Build history of the part. All positions in model axes, mm. A direction names the side the tool comes from. Round coordinates to 2 decimals unless told otherwise and drop trailing zeros. Loops run counter-clockwise (first coordinate to the right, second up) from the corner with the lowest first, then second, coordinate; pieces in that order, holes last.
from build123d import *

# Parameters (mm, degrees)
SKETCH1_R           = 5
SKETCH1_R_2         = 1.5
BOSS_EXTRUDE1_DEPTH = 3
BOSS_EXTRUDE2_START = -3
BOSS_EXTRUDE2_DEPTH = 3
CUT_EXTRUDE2_DEPTH  = 65.81382707
CUT_EXTRUDE3_START  = -10
CUT_EXTRUDE3_DEPTH  = 10


with BuildPart() as part:
    # Sketch1 → Boss-Extrude1 (new body)
    # profile 1 of 3: a face of its own
    with BuildSketch(Plane(origin=(0, 0, 0), x_dir=(0, 0, -1), z_dir=(1, 0, 0))):
        with Locations((5, 5)):
            Circle(SKETCH1_R)
        with Locations((5, 5)):
            Circle(SKETCH1_R_2, mode=Mode.SUBTRACT)
    # profile 2 of 3: a face of its own
    with BuildSketch(Plane(origin=(0, 0, 0), x_dir=(0, 0, -1), z_dir=(1, 0, 0))):
        with BuildLine():
            ThreePointArc((10, 5), (8.535533906, 1.464466094), (5, 0))
            Line((5, 0), (27, 0))
            ThreePointArc((27, 0), (22, 5), (27, 10))
            Line((27, 10), (5, 10))
            ThreePointArc((5, 10), (8.535533906, 8.535533906), (10, 5))
        make_face()
    # profile 3 of 3: a face of its own
    with BuildSketch(Plane(origin=(0, 0, 0), x_dir=(0, 0, -1), z_dir=(1, 0, 0))):
        with Locations((27, 5)):
            Circle(SKETCH1_R)
        with Locations((27, 5)):
            Circle(SKETCH1_R_2, mode=Mode.SUBTRACT)
    extrude(amount=BOSS_EXTRUDE1_DEPTH)

    # Sketch2 → Boss-Extrude2 (add)
    with BuildSketch(Plane(origin=(3, 0, 0), x_dir=(0, 0, -1), z_dir=(1, 0, 0)).offset(BOSS_EXTRUDE2_START)):
        with BuildLine():
            ThreePointArc((27, 10), (29.694507461, 9.21184396), (31.53953799, 7.095851816))
            Line((31.53953799, 7.095851816), (31.610157793, 7.262674791))
            Line((31.610157793, 7.262674791), (44.585599673, 12.519851602))
            Line((44.585599673, 12.519851602), (51.097249205, 9.763328363))
            Line((51.097249205, 9.763328363), (60.365421977, 13.518454657))
            Line((60.365421977, 13.518454657), (56.610295683, 22.786627428))
            Line((56.610295683, 22.786627428), (25.051124858, 10))
            Line((25.051124858, 10), (27, 10))
        make_face()
        Polygon((60.365421977, 13.518454657), (51.097249205, 9.763328363), (51.333822162, 9.179433479), (60.601994933, 12.934559772), align=None)
    extrude(amount=BOSS_EXTRUDE2_DEPTH)

    # Sketch4 → Cut-Extrude2 (cut, through all)
    with BuildSketch(Plane(origin=(3, 0, 0), x_dir=(0, 0, -1), z_dir=(1, 0, 0))):
        Polygon((56.610295683, 22.786627428), (51.684261855, 20.790777803), (58.606145308, 17.8605936), align=None)
    extrude(amount=-CUT_EXTRUDE2_DEPTH, mode=Mode.SUBTRACT)

    # Sketch5 → Cut-Extrude3 (cut)
    with BuildSketch(Plane(origin=(3, 0, 0), x_dir=(0, 0, -1), z_dir=(1, 0, 0)).offset(CUT_EXTRUDE3_START)):
        with BuildLine():
            ThreePointArc((27, 0), (31.21184396, 2.305492539), (31.53953799, 7.095851816))
            Line((31.53953799, 7.095851816), (29.583779735, 2.664986829))
            Line((29.583779735, 2.664986829), (25.539598719, 0))
            Line((25.539598719, 0), (27, 0))
        make_face()
        Polygon((52.260639439, 9.554946108), (51.097249205, 9.763328363), (51.333822162, 9.179433479), align=None)
        Polygon((52.95088376, 10.514353622), (52.260639439, 9.554946108), (54.114273993, 10.305971367), align=None)
        Polygon((54.804518314, 11.265378881), (54.114273993, 10.305971367), (55.967908548, 11.056996626), align=None)
        Polygon((56.658152868, 12.01640414), (55.967908548, 11.056996626), (57.821543102, 11.808021884), align=None)
        Polygon((58.511787422, 12.767429398), (57.821543102, 11.808021884), (59.675177656, 12.559047143), align=None)
        Polygon((60.365421977, 13.518454657), (59.675177656, 12.559047143), (60.601994933, 12.934559772), align=None)
    extrude(amount=CUT_EXTRUDE3_DEPTH, mode=Mode.SUBTRACT)


solid = part.part
(1) Pull direction Z, two halves, no side cores. Call faces 1 (the face through (1.48, 11.16, -47.8)), 2 (the face through (1, 0, -15)), 3 (the face through (1.479, 15.659, -59.498)): +Z half, -Z half, draft (parallel to the pull), parting line (faces both ways), or undercut.
Responses:
face 1: undercut
face 2: draft
face 3: -Z half
(2) Probe line 1 (Z direction, x = 0.5, y = 4.5); line 2 (Y direction, x = 1.35, z = -5); line 3 (Y direction, x = 1.8, z = -22). List the from-to ranges inside material, lowest first.
Responses:
line 1: z = -30.39 to -28.41, -25.59 to -6.41, -3.59 to -0.03
line 2: y = 0 to 3.5, 6.5 to 10
line 3: y = 0 to 10
(3) Pin check, flat tips, straight feed: P1, Ø1, axis at x = 2.5, z = -37, coming from the +Y side; P2, Ø1.5, axis at x = 1, y = 16, coming from the -Z side. Stop position of each tip, or through.
Responses:
P1: stops at y = 15.04
P2: stops at z = -59.66
(4) Slice it at D-D on z = -38.5. List the corners of the cut face in (x, y).
Responses:
outline: (0, 10.05) - (3, 10.05) - (3, 15.45) - (0, 15.45) - close
(5) Which spindle directions (+Z, -Z, +X, -X, +Y, -Y) get a long thin tool onto all of the face, cutting with end or side? Do faces 4 (the face through (1.48, 5.07, -25.5)), 5 (the face through (1.479, 9.854, -38.007)). Say none if no direction does.
Responses:
face 4: +X, -X
face 5: +X, -X, -Y
(6) Slice it at B-B on z = -27. List the corners of the cut face in (x, y).
Responses:
outline: (0, 0.96) - (3, 0.96) - (3, 3.5) - (0, 3.5) - close; (0, 6.5) - (3, 6.5) - (3, 10.79) - (0, 10.79) - close
(7) Slice it at A-A on x = 2.3. List the corners of the cut face in (y, z), plus the area to 3 significant figures.
Responses:
outline: (0, -25.54) - (2.66, -29.58) - (7.1, -31.54) - (7.26, -31.61) - (12.52, -44.59) - (9.76, -51.1) - (9.55, -52.26) - (10.51, -52.95) - (10.31, -54.11) - (11.27, -54.8) - (11.06, -55.97) - (12.02, -56.66) - (11.81, -57.82) - (12.77, -58.51) - (12.56, -59.68) - (13.52, -60.37) - (17.86, -58.61) - (20.79, -51.68) - (10, -25.05) - (10, -5) arc R5 ccw to (0, -5) - close; hole circle Ø3 at (5, -27); hole circle Ø3 at (5, -5)
area: 476 mm2
(8) Slice it at C-C on y = 5. List the corners of the cut face in (x, z).
Responses:
outline: (0, -30.61) - (3, -30.61) - (3, -28.5) - (0, -28.5) - close; (0, -25.5) - (3, -25.5) - (3, -6.5) - (0, -6.5) - close; (0, -3.5) - (3, -3.5) - (3, 0) - (0, 0) - close
